Here's how the part is built. I have some questions about the finished solid (model axes, mm). Round coordinates to 2 decimals unless told otherwise and drop trailing zeros. Loops run counter-clockwise (first coordinate to the right, second up) from the corner with the lowest first, then second, coordinate; pieces in that order, holes last. Notation, with made-up numbers: M -2.75,-21.5 L 30.25,-21.5 A33 ccw 30.25,6.5 Z; hole C 3.25,64 d4. An arc over 180 degrees is marked long. Answer as a JSON object with one key per item and string values.
from build123d import *

# Parameters (mm, degrees)
SKETCH1_W                      = 900
SKETCH1_H                      = 260
BOSS_EXTRUDE1_DEPTH            = 40
F_17_0_17_DIAMETER_HOLE1_D     = 17
F_17_0_17_DIAMETER_HOLE1_DEPTH = 42
F_17_0_17_DIAMETER_HOLE1_TIP   = 5.107315262
CHAMFER1_SIZE                  = 20


with BuildPart() as part:
    # Sketch1 → Boss-Extrude1 (new body)
    with BuildSketch(Plane.XY):
        Rectangle(SKETCH1_W, SKETCH1_H)
    extrude(amount=BOSS_EXTRUDE1_DEPTH)

    # Ø17.0 (17) Diameter Hole1
    with Locations(Plane.XY.offset(40)):
        with Locations((-370, 100), (-140, 100), (-370, -100), (-140, -100), (140, -100), (370, -100), (140, 100), (370, 100)):
            Hole(F_17_0_17_DIAMETER_HOLE1_D / 2, depth=F_17_0_17_DIAMETER_HOLE1_DEPTH)
            with Locations((0, 0, -(F_17_0_17_DIAMETER_HOLE1_DEPTH + F_17_0_17_DIAMETER_HOLE1_TIP / 2))):  # 118° drill point
                Cone(0, F_17_0_17_DIAMETER_HOLE1_D / 2, F_17_0_17_DIAMETER_HOLE1_TIP, mode=Mode.SUBTRACT)

    # Chamfer1
    chamfer1_edges = [part.edges().sort_by_distance(p)[0] for p in [
        (-450, 130, 20),
        (450, 130, 20),
        (450, -130, 20),
        (-450, -130, 20),
    ]]
    chamfer(chamfer1_edges, length=CHAMFER1_SIZE)


solid = part.part
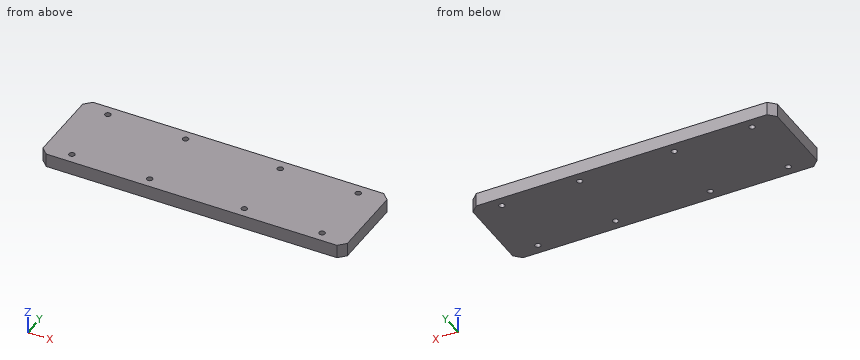
Item 1: I want a section at B-B on y = 100. List the corners of the cut face in (x, z) for me.
Solution:
{"outline": "M -450,0 L -378.5,0 L -378.5,40 L -450,40 Z; M -361.5,0 L -148.5,0 L -148.5,40 L -361.5,40 Z; M -131.5,0 L 131.5,0 L 131.5,40 L -131.5,40 Z; M 148.5,0 L 361.5,0 L 361.5,40 L 148.5,40 Z; M 378.5,0 L 450,0 L 450,40 L 378.5,40 Z"}
Item 2: If I drill on L1, parallel to Y at x = -370, z = 31; L2, parallel to X at y = -107, z = 26; L3, parallel to Y at x = 142, z = 2, over which ranges is the centre line in solid material (lowest first)? Write a range as from..to.
Solution:
{"L1": "y = -130..-108.5, -91.5..91.5, 108.5..130", "L2": "x = -450..-374.82, -365.18..-144.82, -135.18..135.18, 144.82..365.18, 374.82..450", "L3": "y = -130..-108.26, -91.74..91.74, 108.26..130"}
Item 3: I want a section at A-A on x = -140. List the corners of the cut face in (y, z) for me.
Solution:
{"outline": "M -130,0 L -108.5,0 L -108.5,40 L -130,40 Z; M -91.5,0 L 91.5,0 L 91.5,40 L -91.5,40 Z; M 108.5,0 L 130,0 L 130,40 L 108.5,40 Z"}
Item 4: For P1, Ø15.5, axis at x = -140, y = 100, coming from the -Z side, with a flat end and sliding along its axis, tell me the tip position at first contact or that it passes through.
Solution:
{"P1": "passes through"}
